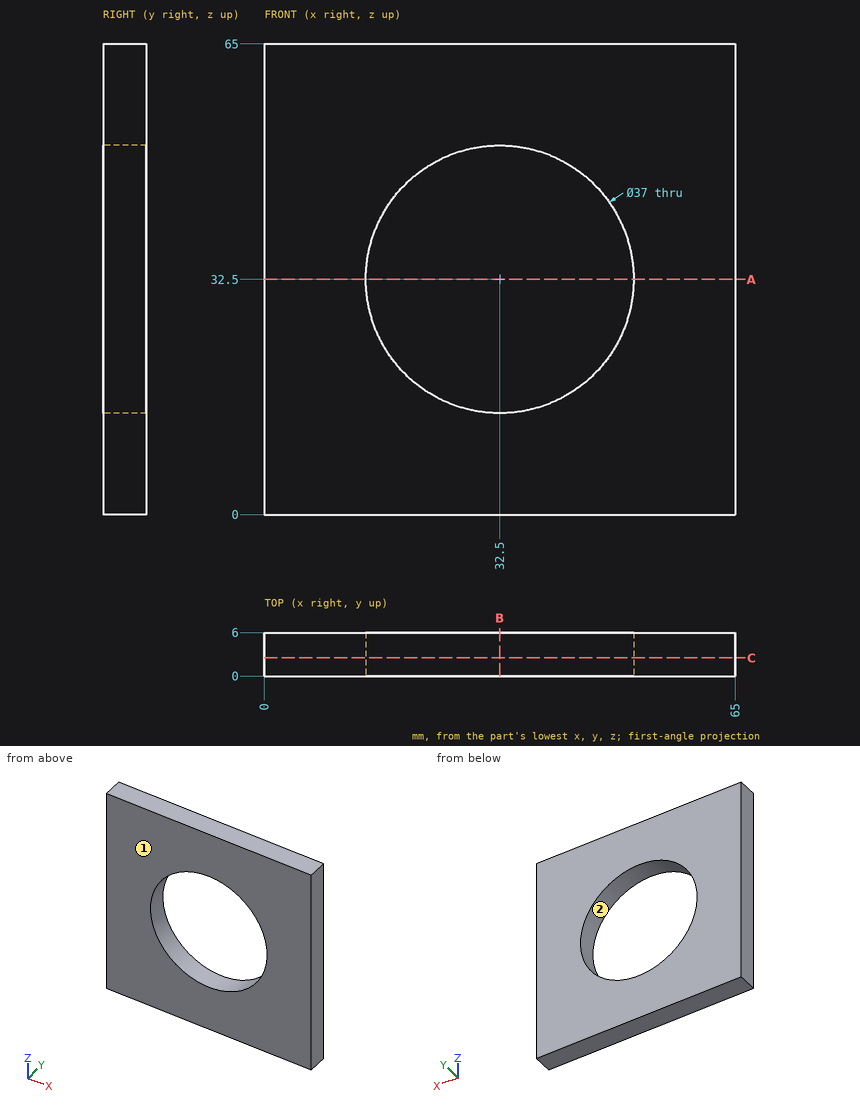
Design review of the part shown in the three views and the two pictorial views. Dimensions are in mm from the part's minimum x, y and z. Coordinates: 2 decimals unless noted, no trailing zeros. Loops run counter-clockwise (first coordinate to the right, second up) from the corner with the lowest first, then second, coordinate; pieces in that order, holes last. Notation, with made-up numbers: M 61,22 L 68,22 A26 ccw 68,38 Z; hole C 72,66 d7. An arc over 180 degrees is marked long. Put each result on its own line as item: value. Start each with the question number.
Q1. Add section B-B (x = 32.5). Write out the cut boundary in (y, z), and give its area (3 significant figures).
Q2. The part is to be moulded in two halves that separate along Z. For the marked faces 1 and 2, say which applies: +Z half, -Z half, draft (parallel to the pull), parting line (faces both ways), or undercut.
Q3. Add section C-C (y = 2.5). Write out the cut boundary in (x, z).
Q4. Wall thickness on line 1 (X direction, y = 3.5, z = 32.5); line 2 (X direction, y = 1.9, z = 38.5); line 3 (Z direction, x = 30.5, y = 4.3): over which ranges is each line inside the solid? List them lowest first.
Q5. Add section A-A (z = 32.5). Write out the cut boundary in (x, y).
Q6. Clearance check with a flat-ended pin moving along its axis: pin 1 (22 mm diameter, centred on x = 32.5, z = 32.5, fed in from +Y). State where the tip first meets the part, or that it passes through.
Answers:
1. outline: M 0,0 L 6,0 L 6,14 L 0,14 Z; M 0,51 L 6,51 L 6,65 L 0,65 Z
1. area: 168 mm^2
2. face 1: draft
2. face 2: undercut
3. outline: M 0,0 L 65,0 L 65,65 L 0,65 Z; hole C 32.5,32.5 d37
4. line 1: x = 0 to 14, 51 to 65
4. line 2: x = 0 to 15, 50 to 65
4. line 3: z = 0 to 14.11, 50.89 to 65
5. outline: M 0,0 L 14,0 L 14,6 L 0,6 Z; M 51,0 L 65,0 L 65,6 L 51,6 Z
6. pin 1: passes through
